```python
from build123d import *

# Parameters (mm, degrees)
SKETCH_1_W          = 27
SKETCH_1_H          = 16
EXTRUDE_1_DEPTH     = 4
SKETCH_2_R          = 0.75
SKETCH_2_R_2        = 1.59
CUT_EXTRUDE_2_DEPTH = 4
CUT_EXTRUDE_3_DEPTH = 4


with BuildPart() as part:
    # 草图1 → 凸台-拉伸1 (new body)
    with BuildSketch(Plane.XY):
        with Locations((3.898916968, -3.881768953)):
            Rectangle(SKETCH_1_W, SKETCH_1_H)
    extrude(amount=EXTRUDE_1_DEPTH)

    # 草图2 → 切除-拉伸2 (cut)
    with BuildSketch(Plane.XY.offset(4)):
        with Locations((1.199905932, -1.781578746)):
            Circle(SKETCH_2_R)
        with Locations((1.122511443, -6.056778774)):
            Circle(SKETCH_2_R)
        with Locations((9.465404763, -4.069510677)):
            Circle(SKETCH_2_R_2)
    extrude(amount=-CUT_EXTRUDE_2_DEPTH, mode=Mode.SUBTRACT)

    # 草图3 → 切除-拉伸3 (cut)
    with BuildSketch(Plane.XY.offset(4)):
        with BuildLine():
            Line((6.931862452, -2.481455291), (9.464184068, -2.479511145))
            ThreePointArc((9.464184068, -2.479511145), (7.875405231, -4.070731371), (9.466625457, -5.659510208))
            Line((9.466625457, -5.659510208), (6.934303841, -5.661454354))
            ThreePointArc((6.934303841, -5.661454354), (5.343083615, -4.072675517), (6.931862452, -2.481455291))
        make_face()
        with BuildLine():
            Line((-1.276445305, -7.332757851), (0.601227077, -5.517554692))
            ThreePointArc((0.601227077, -5.517554692), (0.583287361, -6.578063139), (1.643795809, -6.596002856))
            Line((1.643795809, -6.596002856), (-0.233876574, -8.411206015))
            ThreePointArc((-0.233876574, -8.411206015), (-1.294385021, -8.393266299), (-1.276445305, -7.332757851))
        make_face()
        with BuildLine():
            Line((-1.145979965, -0.556904877), (0.678621567, -2.320802827))
            ThreePointArc((0.678621567, -2.320802827), (0.660681851, -1.26029438), (1.721190298, -1.242354664))
            Line((1.721190298, -1.242354664), (-0.103411234, 0.521543286))
            ThreePointArc((-0.103411234, 0.521543286), (-1.163919681, 0.50360357), (-1.145979965, -0.556904877))
        make_face()
    extrude(amount=-CUT_EXTRUDE_3_DEPTH, mode=Mode.SUBTRACT)


solid = part.part
```
Build history of the part. All positions in model axes, mm. A direction names the side the tool comes from. Coordinates: 2 decimals unless noted, no trailing zeros. Order: outer loops, then holes, each group sorted by start corner. A loop starts at its lowest first (then second) coordinate and runs counter-clockwise, first axis right, second up. Notation, with made-up numbers: (40.25, 13) -> (86.25, 13) arc R19 cw to (86.25, 47) -> close; hole circle Ø3 at (-7, -37). An arc over 180 degrees is marked (long way). Answer in a Markdown table with one row per item. Add a question column.
Q1. Mould opens along Y. For faces 1 (the face through (4, -4, 0)), 2 (the face through (-0.246, -1.427, 2.028)), 3 (the face through (4, -11.882, 2)) say: +Y half, -Y half, draft (parallel to the pull), parting line (faces both ways), or undercut.
Q2. Wall check: line 1 along Y through (x, z) = (7.75, 2); line 2 along X through (y, z) = (-7.25, 3); line 3 along X through (y, z) = (-4.25, 1.6). Give the ranges that are in metal, low to high. Write a range as [from, to].
Q3. Drop a flat-ended pin along its axis: pin 1 (1.5 mm diameter, centred on x = 14.5, y = -0.5, fed in from -Z). Give the stop position or say it passes through.
Q4. Band-saw the part on B-B, the plane y = -1.5. List the corners of the cut face in (x, z).
Q5. Band-saw the part on A-A, the plane z = 2.4. List the corners of the cut face in (x, y).
Q6. Band-saw the part on C-C, the plane x = 8.75. List the corners of the cut face in (y, z).
Q7. Band-saw the part on D-D, the plane x = -0.75. List the corners of the cut face in (y, z).
Q8. Which spindle directions (+Z, -Z, +X, -X, +Y, -Y) get a long thin tool onto all of the face, cutting with end or side? Do faces 4 (the face through (-9.601, -4, 2)), 5 (the face through (11.055, -4.103, 2.028)). Say none if no direction does.
Answers follow:
| question | item | result |
|---|---|---|
| 1 | face 1 | draft |
| 1 | face 2 | undercut |
| 1 | face 3 | -Y half |
| 2 | line 1 | [-11.88, -5.66], [-2.48, 4.12] |
| 2 | line 2 | [-9.6, -1.19], [0.97, 17.4] |
| 2 | line 3 | [-9.6, 5.35], [11.05, 17.4] |
| 3 | pin 1 | z = 0 |
| 4 | outline | (-9.6, 0) -> (-0.17, 0) -> (-0.17, 4) -> (-9.6, 4) -> close; (1.9, 0) -> (17.4, 0) -> (17.4, 4) -> (1.9, 4) -> close |
| 5 | outline | (-9.6, -11.88) -> (17.4, -11.88) -> (17.4, 4.12) -> (-9.6, 4.12) -> close; hole (-1.28, -7.33) arc R0.75 ccw to (-0.23, -8.41) -> (1.64, -6.6) arc R0.75 ccw to (0.6, -5.52) -> close; hole (-1.15, -0.56) -> (0.68, -2.32) arc R0.75 ccw to (1.72, -1.24) -> (-0.1, 0.52) arc R0.75 ccw to start; hole (6.93, -5.66) -> (9.47, -5.66) arc R1.59 ccw to (9.46, -2.48) -> (6.93, -2.48) arc R1.59 ccw to start |
| 6 | outline | (-11.88, 0) -> (-5.66, 0) -> (-5.66, 4) -> (-11.88, 4) -> close; (-2.48, 0) -> (4.12, 0) -> (4.12, 4) -> (-2.48, 4) -> close |
| 7 | outline | (-11.88, 0) -> (-8.62, 0) -> (-8.62, 4) -> (-11.88, 4) -> close; (-6.82, 0) -> (-0.94, 0) -> (-0.94, 4) -> (-6.82, 4) -> close; (0.72, 0) -> (4.12, 0) -> (4.12, 4) -> (0.72, 4) -> close |
| 8 | face 4 | +Z, -Z, -X, +Y, -Y |
| 8 | face 5 | +Z, -Z |
